```python
from build123d import *

# Parameters (mm, degrees)
SKETCH_1_R          = 12
EXTRUDE_1_DEPTH     = 10
CHAMFER_1_SIZE      = 0.5
CUT_EXTRUDE_1_DEPTH = 8


with BuildPart() as part:
    # 草图1 → 凸台-拉伸1 (new body)
    with BuildSketch(Plane.XY):
        Circle(SKETCH_1_R)
    extrude(amount=EXTRUDE_1_DEPTH)

    # 倒角1
    chamfer_1_edges = [part.edges().sort_by_distance(p)[0] for p in [
        (-12, 0, 0),
        (-12, 0, 10),
    ]]
    chamfer(chamfer_1_edges, length=CHAMFER_1_SIZE)

    # 草图2 → 切除-拉伸1 (cut)
    with BuildSketch(Plane(origin=(0, 0, 0), x_dir=(-1, 0, 0), z_dir=(0, 0, -1))):
        Polygon((0, -3.464101615), (3, -1.732050808), (3, 1.732050808), (0, 3.464101615), (-3, 1.732050808), (-3, -1.732050808), align=None)
    extrude(amount=-CUT_EXTRUDE_1_DEPTH, mode=Mode.SUBTRACT)


solid = part.part
```
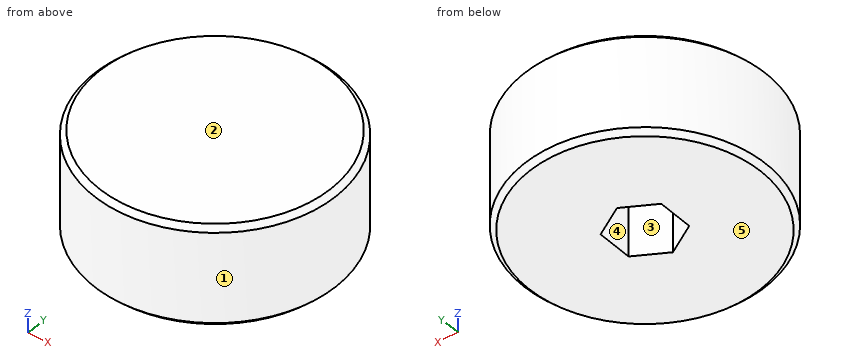
Geometry check sheet. Reference: the model listing, model coordinates, mm. Face numbers are marked on the shaded views. A direction names the side the tool comes from. Coordinates: 2 decimals unless noted, no trailing zeros. Write each loop counter-clockwise with the first axis right and the second up, starting at its lowest first coordinate (ties: lowest second). Pieces come first, ordered by that corner, then holes. Notation, with made-up numbers: M 87.25,15.25 L 102.25,15.25 A12 ccw 102.25,32.25 Z; hole C 25.25,68.5 d4. An arc over 180 degrees is marked long. Use one line per item in the form item = value. Start each with the question number.
1) Release check for a two-part mould opening along Y. For the marked faces 1, 2 and 3 record: pulls with the +Y half, pulls with the -Y half, needs draft (parallel to the pull), parting line crosses it, or undercut.
2) Section check B-B on y = 0. Enter the section's corners in (x, z).
3) Thickness scan on probe 1 along Y at (x, z) = (0.25, 9.5); probe 2 along X at (y, z) = (3, 1.25); probe 3 along Y at (x, z) = (0.25, 6.5). Record the ranges inside material, lowest first. Write a range as from..to.
4) Set-up check for the marked faces 4 and 5: record each of +Z, -Z, +X, -X, +Y, -Y from which the full face is reachable in a straight line by a thin tool's end or side.
5) Go/stop test with flat-tipped pins: pin 1 Ø3 at (x, z) = (-7.5, 8) entering from -Y; pin 2 Ø2 at (y, z) = (-1.5, 6.5) entering from -X. Record where each tip stops, or that it passes through.
6) Section check A-A on z = 4.25. Enter the section's corners in (x, y), and give its area (3 significant figures).
Responses:
q1.face_1 = parting line crosses it
q1.face_2 = needs draft
q1.face_3 = undercut
q2.outline = M -12,0.5 L -11.5,0 L -3,0 L -3,8 L 3,8 L 3,0 L 11.5,0 L 12,0.5 L 12,9.5 L 11.5,10 L -11.5,10 L -12,9.5 Z
q3.probe_1 = -12..12
q3.probe_2 = -11.62..-0.8, 0.8..11.62
q3.probe_3 = -12..-3.32, 3.32..12
q4.face_4 = -Z
q4.face_5 = -Z, +X, -X, +Y, -Y
q5.pin_1 = -10.39
q5.pin_2 = -11.99
q6.outline = C 0,0 d24; hole M -3,-1.73 L 0,-3.46 L 3,-1.73 L 3,1.73 L 0,3.46 L -3,1.73 Z
q6.area = 421 mm2
